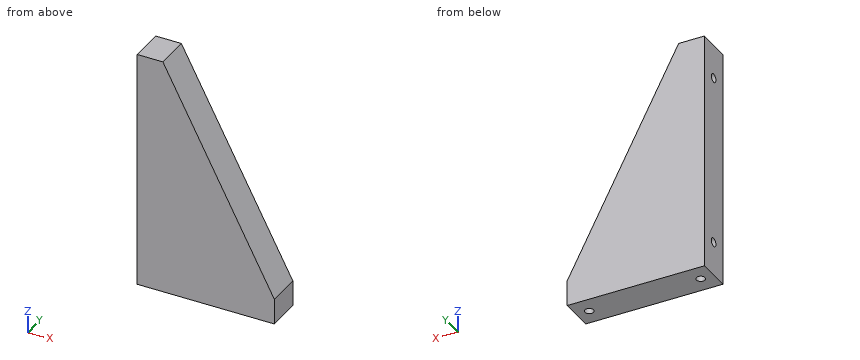
```python
from build123d import *

# Parameters (mm, degrees)
SKETCH_1_W             = 200
SKETCH_1_H             = 140
EXTRUDE_1_DEPTH        = 20
SKETCH_3_OUTSIDE_W     = 250.99
SKETCH_3_OUTSIDE_H     = 190.99
CUT_EXTRUDE_1_DEPTH    = 245.948974278
HOLE_WIZARD_M6_1_D     = 5
HOLE_WIZARD_M6_1_DEPTH = 15
HOLE_WIZARD_M6_1_TIP   = 1.502151548
HOLE_WIZARD_M6_2_D     = 5
HOLE_WIZARD_M6_2_DEPTH = 15
HOLE_WIZARD_M6_2_TIP   = 1.502151548


with BuildPart() as part:
    # 草图1 → 凸台-拉伸1 (new body)
    with BuildSketch(Plane(origin=(0, 0, 0), x_dir=(1, 0, 0), z_dir=(0, 1, 0))):
        with Locations((100, 70)):
            Rectangle(SKETCH_1_W, SKETCH_1_H)
    extrude(amount=EXTRUDE_1_DEPTH)

    # 草图3 outside → 切除-拉伸1 (cut, through all)
    with BuildSketch(Plane(origin=(0, 20, 0), x_dir=(1, 0, 0), z_dir=(0, 1, 0))):
        with Locations((100, 70)):
            Rectangle(SKETCH_3_OUTSIDE_W, SKETCH_3_OUTSIDE_H)
        Polygon((0, 140), (80, 140), (80, 125), (15, 0), (0, 0), align=None, mode=Mode.SUBTRACT)
    extrude(amount=-CUT_EXTRUDE_1_DEPTH, mode=Mode.SUBTRACT)

    # M6 螺纹孔1
    with Locations(Plane.ZY):
        with Locations((-120, 10), (-20, 10)):
            Hole(HOLE_WIZARD_M6_1_D / 2, depth=HOLE_WIZARD_M6_1_DEPTH)
            with Locations((0, 0, -(HOLE_WIZARD_M6_1_DEPTH + HOLE_WIZARD_M6_1_TIP / 2))):  # 118° drill point
                Cone(0, HOLE_WIZARD_M6_1_D / 2, HOLE_WIZARD_M6_1_TIP, mode=Mode.SUBTRACT)

    # M6 螺纹孔2
    with Locations(Plane(origin=(0, 0, -140), x_dir=(-1, 0, 0), z_dir=(0, 0, -1))):
        with Locations((-72.5, 10), (-7.5, 10)):
            Hole(HOLE_WIZARD_M6_2_D / 2, depth=HOLE_WIZARD_M6_2_DEPTH)
            with Locations((0, 0, -(HOLE_WIZARD_M6_2_DEPTH + HOLE_WIZARD_M6_2_TIP / 2))):  # 118° drill point
                Cone(0, HOLE_WIZARD_M6_2_D / 2, HOLE_WIZARD_M6_2_TIP, mode=Mode.SUBTRACT)


solid = part.part
```
Build history of the part. All positions in model axes, mm. Coordinates: 2 decimals unless noted, no trailing zeros. Order: outer loops, then holes, each group sorted by start corner. A loop starts at its lowest first (then second) coordinate and runs counter-clockwise, first axis right, second up. Notation, with made-up numbers: (-21.75, 66) -> (30.25, 66) arc R32 ccw to (30.25, 95) -> close; hole circle Ø9 at (-13.75, 13.25). An arc over 180 degrees is marked (long way). Answer in a Markdown table with one row per item. Add a question column.
Q1. Band-saw the part on B-B, the plane y = 16.25. List the corners of the cut face in (x, z).
Q2. Band-saw the part on A-A, the plane z = -38. List the corners of the cut face in (x, y), then the cut area to 3 significant figures.
Q3. Wall check: line 1 along X through (y, z) = (10, -129.25); line 2 along Z through (x, y) = (3.5, 10); line 3 along Y through (x, z) = (72.5, -130.75). Give the ranges that are in metal, low to high. Write a range as [from, to].
Q4. Band-saw the part on C-C, the plane x = 27. List the corners of the cut face in (y, z), then the cut area to 3 significant figures.
Q5. Drop flat-ended pins along their axis: pin 1 (3 mm diameter, centred on x = 72.5, y = 10, fed in from +Z); pin 2 (8 mm diameter, centred on y = 10, z = -120, fed in from +X); pin 3 (1 mm diameter, centred on y = 14, z = -31, fed in from +X). Give the stop position or say it passes through.
Answers follow:
| question | item | result |
|---|---|---|
| 1 | outline | (0, -140) -> (80, -140) -> (80, -125) -> (15, 0) -> (0, 0) -> close |
| 2 | outline | (0, 0) -> (34.76, 0) -> (34.76, 20) -> (0, 20) -> close |
| 2 | area | 695 mm^2 |
| 3 | line 1 | [0, 5], [10, 70], [75, 80] |
| 3 | line 2 | [-140, -122.5], [-117.5, -22.5], [-17.5, 0] |
| 3 | line 3 | [0, 7.5], [12.5, 20] |
| 4 | outline | (0, -140) -> (20, -140) -> (20, -23.08) -> (0, -23.08) -> close |
| 4 | area | 2,340 mm^2 |
| 5 | pin 1 | z = -107.69 |
| 5 | pin 2 | x = 79.48 |
| 5 | pin 3 | x = 31.38 |
